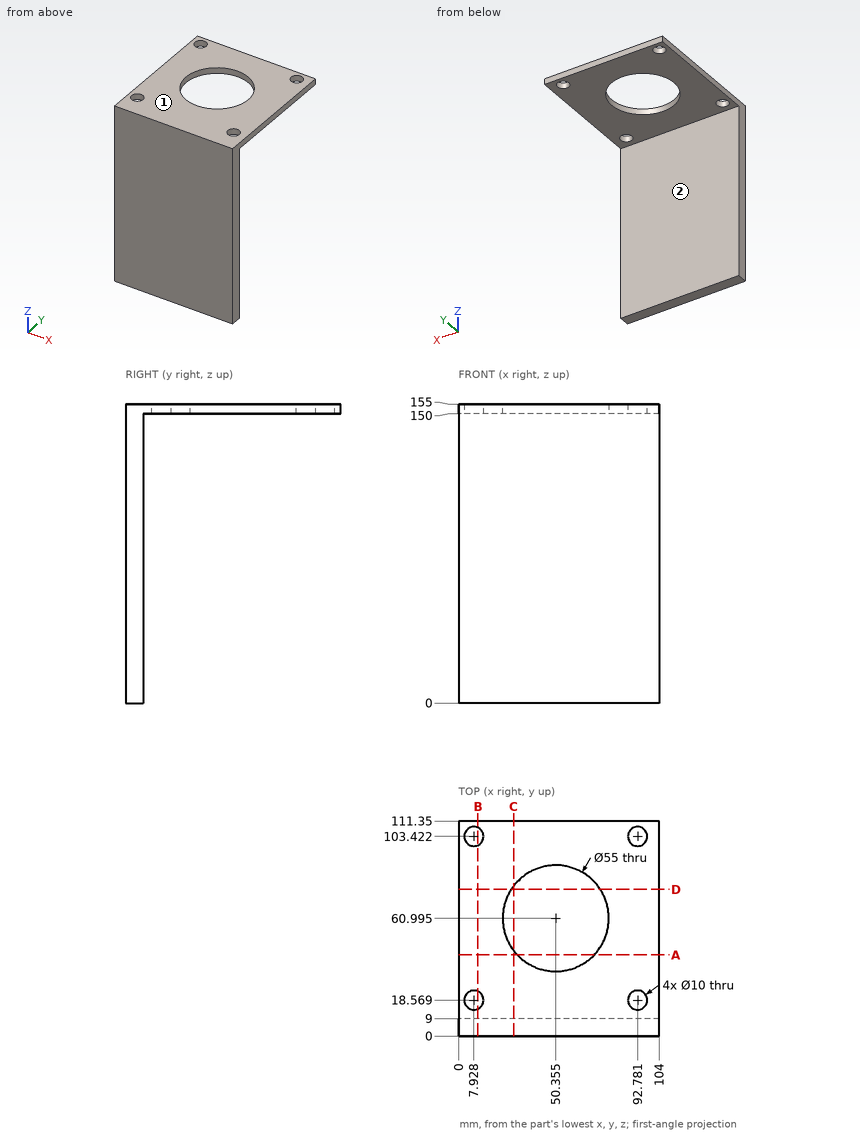
Here's the drawing with two shaded views (mm, measured from the low corner). I have some questions. A direction names the side the tool comes from. Round coordinates to 2 decimals unless told otherwise and drop trailing zeros. Order: outer loops, then holes, each group sorted by start corner. A loop starts at its lowest first (then second) coordinate and runs counter-clockwise, first axis right, second up. Notation, with made-up numbers: M 0.5,-38.75 L 39.5,-38.75 A30 cw 39.5,0.25 Z; hole C 31,-15 d1. An arc over 180 degrees is marked long. Use CSV: the item, a comma, the result in double quotes.
1) I need wall thicknesses on line 1 along Y through (x, z) = (25, 128); line 2 along Z through (x, y) = (17, 99). Which ranges of each line are inside material? Lowest first, please. Write a range as [from, to].
Taken from the geometry:
line 1,"[0, 9]"
line 2,"[150, 155]"
2) I want a section at D-D (y = 76). List the corners of the cut face in (x, z) for me.
Taken from the geometry:
outline,"M 0,150 L 27.31,150 L 27.31,155 L 0,155 Z; M 73.4,150 L 104,150 L 104,155 L 73.4,155 Z"
3) On a 3-axis mill with a long thin cutter (end or side, diameter ignored), from which of +Z, -Z, +X, -X, +Y, -Y can I reach the whole of each face in a straight line? I mean the marked faces 1 and 2. Say none if no direction works.
Taken from the geometry:
face 1,"+Z, +X, -X, +Y, -Y"
face 2,"-Z, +X, -X, +Y"
4) I want a section at A-A (y = 42). List the corners of the cut face in (x, z) for me.
Taken from the geometry:
outline,"M 0,150 L 30.47,150 L 30.47,155 L 0,155 Z; M 70.24,150 L 104,150 L 104,155 L 70.24,155 Z"
5) I want a section at B-B (x = 10). List the corners of the cut face in (y, z) for me.
Taken from the geometry:
outline,"M 0,0 L 9,0 L 9,150 L 14.02,150 L 14.02,155 L 0,155 Z; M 23.12,150 L 98.87,150 L 98.87,155 L 23.12,155 Z; M 107.97,150 L 111.35,150 L 111.35,155 L 107.97,155 Z"
6) I want a section at C-C (x = 28.5). List the corners of the cut face in (y, z) for me, then the cut area to 3 significant figures.
Taken from the geometry:
outline,"M 0,0 L 9,0 L 9,150 L 44.3,150 L 44.3,155 L 0,155 Z; M 77.69,150 L 111.35,150 L 111.35,155 L 77.69,155 Z"
area,"1,740 mm^2"
7) I'm going to push flat-ended pins straight in: P1, Ø9, axis at x = 7.93, y = 18.57, coming from the +Z side; P2, Ø6, axis at x = 86.5, z = 104.5, coming from the +Y side; P3, Ø16, axis at x = 92.78, y = 18.57, coming from the -Z side; P4, Ø1.5, axis at x = 53, z = 43.5, coming from the -Y side. Where does each tip first touch, or does it pass through?
Taken from the geometry:
P1,"through"
P2,"y = 9"
P3,"z = 150"
P4,"y = 0"
